Model file for the job. Use its own axes, mm. Coordinates: 2 decimals unless noted, no trailing zeros. Order: outer loops, then holes, each group sorted by start corner. A loop starts at its lowest first (then second) coordinate and runs counter-clockwise, first axis right, second up. Notation, with made-up numbers: (-19.75, -13) -> (4.25, -13) arc R17 ccw to (4.25, 20) -> close; hole circle Ø6 at (-6.5, -27.75). An arc over 180 degrees is marked (long way). Use CSV: the item, a comma, the result in double quotes. Start each with the question number.
(1) Pin check, flat tip, straight feed: pin 1 Ø4 at (y, z) = (55, 3.5) entering from -X. Stop position of the tip, or through.
(2) Cut at A-A on z = 13.5. Write the cut outline in (x, y).
(3) Cut at C-C on y = 40.5. Write the cut outline in (x, z).
(4) Cut at B-B on x = -3. Write the cut outline in (y, z).
(5) Probe L1, parallel to X at y = 28, z = 6; L2, parallel to X at y = 17.5, z = 3.75. List the from-to ranges inside material, lowest first.
```python
from build123d import *

# Parameters (mm, degrees)
GUSSET_PLATE_15MM_DEPTH = 15
EDGE_CHAMFER_10X45_SIZE = 10


with BuildPart() as part:
    # Gusset Profile Sketch → Gusset Plate 15mm (new body)
    with BuildSketch(Plane.XY):
        Polygon((0, 0), (-50, 0), (-7.128129211, 160), (0, 160), align=None)
    extrude(amount=GUSSET_PLATE_15MM_DEPTH)

    # Edge Chamfer 10x45
    edge_chamfer_10x45_edges = [part.edges().sort_by_distance(p)[0] for p in [
        (0, 0, 7.5),
    ]]
    chamfer(edge_chamfer_10x45_edges, length=EDGE_CHAMFER_10X45_SIZE)


solid = part.part
```
Outcome:
1,pin 1,"x = -35.8"
2,outline,"(-50, 0) -> (-10, 0) -> (0, 10) -> (0, 160) -> (-7.13, 160) -> close"
3,outline,"(-39.15, 0) -> (0, 0) -> (0, 15) -> (-39.15, 15) -> close"
4,outline,"(7, 0) -> (160, 0) -> (160, 15) -> (7, 15) -> close"
5,L1,"-42.5 to 0"
5,L2,"-45.31 to 0"
